CAD build for the part. Positions are in the model's coordinates, mm. Coordinates: 2 decimals unless noted, no trailing zeros. Write each loop counter-clockwise with the first axis right and the second up, starting at its lowest first coordinate (ties: lowest second). Pieces come first, ordered by that corner, then holes. Notation, with made-up numbers: (17, -13.5) -> (76, -13.5) arc R7 cw to (76, -5.5) -> close; hole circle Ø11 at (57.25, 59). An arc over 180 degrees is marked (long way). Answer as CSV lines item,"result".
```python
from build123d import *

# Parameters (mm, degrees)
SKETCH3_R           = 14.224
BOSS_EXTRUDE1_DEPTH = 7


with BuildPart() as part:
    # Sketch3 → Boss-Extrude1 (new, symmetric)
    with BuildSketch(Plane(origin=(0, 0, 0), x_dir=(1, 0, 0), z_dir=(0, 1, 0))):
        Polygon((19.556, 140.716), (35.306, 124.966), (35.306, -173.734), (19.556, -189.484), (-53.594, -189.484), (-53.594, 140.716), align=None)
        with Locations(Location((0, 0, 0), (0, 0, 270))):
            Circle(SKETCH3_R, mode=Mode.SUBTRACT)
    extrude(amount=BOSS_EXTRUDE1_DEPTH, both=True)


solid = part.part
```
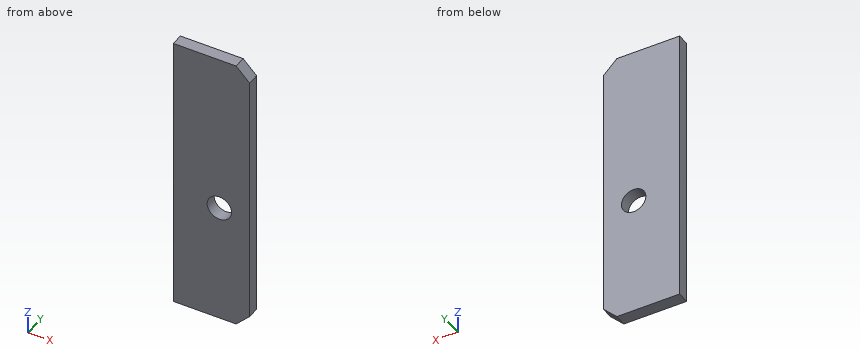
Item 1: Saw through at C-C on z = 0. Give the cut face in (x, y), and give its area (3 significant figures).
Answer below:
outline,"(-53.59, -7) -> (-14.22, -7) -> (-14.22, 7) -> (-53.59, 7) -> close; (14.22, -7) -> (35.31, -7) -> (35.31, 7) -> (14.22, 7) -> close"
area,"846 mm2"
Item 2: Flat gauge pin, fed straight in: pin 1 (2 mm diameter, centred on x = 22, y = 3.5, fed in from +Z). Where does the tip first touch, or does it go through?
Answer below:
pin 1,"stops at z = 188.04"
Item 3: Saw through at B-B on y = 2.5. Give the cut face in (x, z), and give its area (3 significant figures).
Answer below:
outline,"(-53.59, -140.72) -> (19.56, -140.72) -> (35.31, -124.97) -> (35.31, 173.73) -> (19.56, 189.48) -> (-53.59, 189.48) -> close; hole circle Ø28.45 at (0, 0)"
area,"28,500 mm2"
Item 4: Wall check: line 1 (X direction, y = -1, z = 0); line 2 (Z direction, x = 12, y = 2.75); line 3 (Z direction, x = 11.5, y = -5). Give the ranges that are in metal, low to high. Write a range as from..to.
Answer below:
line 1,"x = -53.59..-14.22, 14.22..35.31"
line 2,"z = -140.72..-7.64, 7.64..189.48"
line 3,"z = -140.72..-8.37, 8.37..189.48"
Item 5: Saw through at A-A on x = 0. Give the cut face in (y, z), and give its area (3 significant figures).
Answer below:
outline,"(-7, -140.72) -> (7, -140.72) -> (7, -14.22) -> (-7, -14.22) -> close; (-7, 14.22) -> (7, 14.22) -> (7, 189.48) -> (-7, 189.48) -> close"
area,"4,220 mm2"
